from build123d import *

# Parameters (mm, degrees)
SKETCH_1_W             = 25
SKETCH_1_H             = 72
SKETCH_1_R             = 7.5
EXTRUDE_1_DEPTH        = 50
HOLE_WIZARD_M4_1_D     = 3.3
HOLE_WIZARD_M4_1_DEPTH = 8.1
HOLE_WIZARD_M4_1_TIP   = 0.991420021
CHAMFER_1_SIZE         = 2


with BuildPart() as part:
    # 草图1 → 凸台-拉伸1 (new body)
    with BuildSketch(Plane.XY):
        Rectangle(SKETCH_1_W, SKETCH_1_H)
        with Locations((0, 22.5)):
            Circle(SKETCH_1_R, mode=Mode.SUBTRACT)
        with Locations((0, -22.5)):
            Circle(SKETCH_1_R, mode=Mode.SUBTRACT)
    extrude(amount=EXTRUDE_1_DEPTH)

    # M4 螺纹孔1
    with Locations(Plane(origin=(12.5, 0, 10), x_dir=(0, 0, 1), z_dir=(1, 0, 0))):
        with Locations((0, 0)):
            Hole(HOLE_WIZARD_M4_1_D / 2, depth=HOLE_WIZARD_M4_1_DEPTH)
            with Locations((0, 0, -(HOLE_WIZARD_M4_1_DEPTH + HOLE_WIZARD_M4_1_TIP / 2))):  # 118° drill point
                Cone(0, HOLE_WIZARD_M4_1_D / 2, HOLE_WIZARD_M4_1_TIP, mode=Mode.SUBTRACT)

    # 倒角1
    chamfer_1_edges = [part.edges().sort_by_distance(p)[0] for p in [
        (12.5, -36, 25),
        (-12.5, -36, 25),
        (-12.5, 36, 25),
        (12.5, 36, 25),
    ]]
    chamfer(chamfer_1_edges, length=CHAMFER_1_SIZE)


solid = part.part
The model under review builds one solid part; all positions refer to its coordinate system, in mm. A direction names the side the tool comes from. Round coordinates to 2 decimals unless told otherwise and drop trailing zeros. Loops run counter-clockwise (first coordinate to the right, second up) from the corner with the lowest first, then second, coordinate; pieces in that order, holes last. Notation, with made-up numbers: (-2, 20) -> (35, 20) arc R8 cw to (35, 32) -> close; hole circle Ø11 at (32.25, -15). An arc over 180 degrees is marked (long way). Write item = value, one per line. Start each with the question number.
Item 1: To check wall thickness, follow L1, parallel to Y at x = 0, z = 20; L2, parallel to Y at x = 10, z = 10; L3, parallel to X at y = -22, z = 34. State the ranges of each line that lie inside material, in increasing order.
Item 2: Take a section at A-A on x = 6.75. Give the boundary of the cut face in (y, z).
Item 3: Take a section at D-D on x = 0.5. Give the boundary of the cut face in (y, z), plus the area to 3 significant figures.
Item 4: For faces 1 (the flat face through (-11.5, -35, 24.7)), 2 (the cylindrical face through (8.393, 0.632, 8.476)), list the 3-axis set-ups (+Z, -Z, +X, -X, +Y, -Y) from which the entire face can be reached by the end or side of a thin tool; tool diameter is ignored.
Item 5: Take a section at B-B on y = -22.5. Give the boundary of the cut face in (x, z).
Item 6: Take a section at C-C on z = 46. Give the boundary of the cut face in (x, y), plus the area to 3 significant figures.
Item 7: Mouldability with a two-part tool opening along X and no side actions: class faces 3 (the cylindrical face through (-0.976, -15.064, 24.65)), 4 (the flat face through (0, 1, 50)), 5 (the flat face through (11.5, 35, 24.7)) as released by +X, released by -X, zero draft, split by the parting line, or undercut.
Result:
q1.L1 = -36 to -30, -15 to 15, 30 to 36
q1.L2 = -36 to -1.65, 1.65 to 36
q1.L3 = -12.5 to -7.48, 7.48 to 12.5
q2.outline = (-36, 0) -> (-25.77, 0) -> (-25.77, 50) -> (-36, 50) -> close; (-19.23, 0) -> (19.23, 0) -> (19.23, 50) -> (-19.23, 50) -> close; (25.77, 0) -> (36, 0) -> (36, 50) -> (25.77, 50) -> close; hole circle Ø3.3 at (0, 10)
q3.outline = (-36, 0) -> (-29.98, 0) -> (-29.98, 50) -> (-36, 50) -> close; (-15.02, 0) -> (15.02, 0) -> (15.02, 50) -> (-15.02, 50) -> close; (29.98, 0) -> (36, 0) -> (36, 50) -> (29.98, 50) -> close
q3.area = 2,100 mm²
q4.face_1 = +Z, -Z, -X, -Y
q4.face_2 = +X
q5.outline = (-12.5, 0) -> (-7.5, 0) -> (-7.5, 50) -> (-12.5, 50) -> close; (7.5, 0) -> (12.5, 0) -> (12.5, 50) -> (7.5, 50) -> close
q6.outline = (-12.5, -34) -> (-10.5, -36) -> (10.5, -36) -> (12.5, -34) -> (12.5, 34) -> (10.5, 36) -> (-10.5, 36) -> (-12.5, 34) -> close; hole circle Ø15 at (0, -22.5); hole circle Ø15 at (0, 22.5)
q6.area = 1,440 mm²
q7.face_3 = undercut
q7.face_4 = zero draft
q7.face_5 = released by +X
